Can you work these out from the drawing? Everything is in mm from the part's minimum corner. Round coordinates to 2 decimals unless told otherwise and drop trailing zeros. Loops run counter-clockwise (first coordinate to the right, second up) from the corner with the lowest first, then second, coordinate; pieces in that order, holes last. Notation, with made-up numbers: M 55.5,-9 L 86.5,-9 A15 cw 86.5,9 Z; hole C 22,48 d7. An arc over 180 degrees is marked long. Use a Markdown table: item, result.
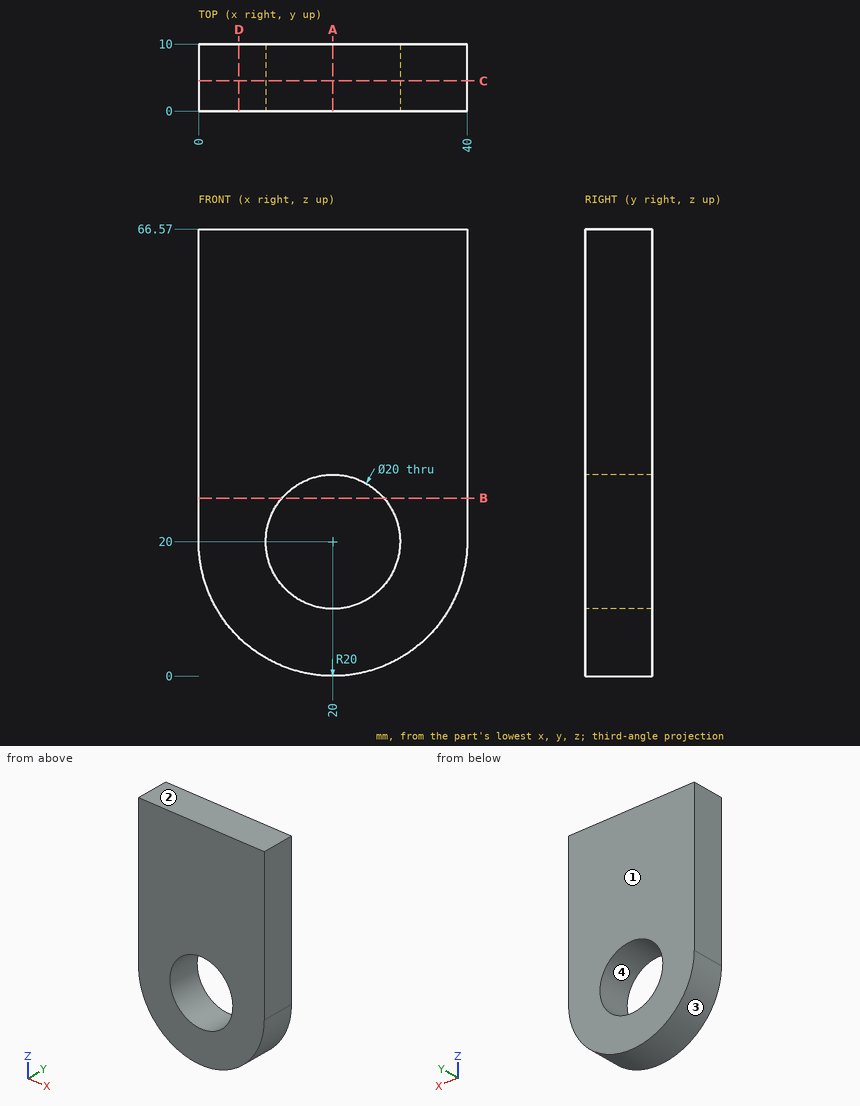
1. For pin 1 Ø1.5 at (y, z) = (2, 18.5) entering from -X; pin 2 Ø4 at (x, y) = (12.5, 6) entering from -Z, each with a flat end and sliding along its axis, tell me the tip position at first contact or that it passes through.
Answer sheet:
| item | result |
|---|---|
| pin 1 | x = 0.01 |
| pin 2 | z = 0.77 |
2. Imagine slicing it at D-D, the plane x = 6. Write out the boundary of the cut face in (y, z).
Answer sheet:
| item | result |
|---|---|
| outline | M 0,5.72 L 10,5.72 L 10,66.57 L 0,66.57 Z |
3. Imagine slicing it at B-B, the plane z = 26.5. Write out the boundary of the cut face in (x, y), then the cut area to 3 significant figures.
Answer sheet:
| item | result |
|---|---|
| outline | M 0,0 L 12.4,0 L 12.4,10 L 0,10 Z; M 27.6,0 L 40,0 L 40,10 L 27.6,10 Z |
| area | 248 mm2 |
4. Imagine slicing it at A-A, the plane x = 20. Write out the boundary of the cut face in (y, z).
Answer sheet:
| item | result |
|---|---|
| outline | M 0,0 L 10,0 L 10,10 L 0,10 Z; M 0,30 L 10,30 L 10,66.57 L 0,66.57 Z |
5. We'd pull the mould along Z, two halves only. Please class the marked faces 1, 2, 3 and 4: +Z half, -Z half, draft (parallel to the pull), parting line (faces both ways), or undercut.
Answer sheet:
| item | result |
|---|---|
| face 1 | draft |
| face 2 | +Z half |
| face 3 | -Z half |
| face 4 | undercut |
6. I need wall thicknesses on probe 1 along X at (y, z) = (6.25, 20); probe 2 along X at (y, z) = (5, 19); probe 3 along Z at (x, y) = (12, 2.5). Which ranges of each line are inside material? Lowest first, please. Write a range as from..to.
Answer sheet:
| item | result |
|---|---|
| probe 1 | 0..10, 30..40 |
| probe 2 | 0.03..10.05, 29.95..39.97 |
| probe 3 | 1.67..14, 26..66.57 |
7. Imagine slicing it at C-C, the plane y = 4.5. Write out the boundary of the cut face in (x, z).
Answer sheet:
| item | result |
|---|---|
| outline | M 0,20 A20 ccw 40,20 L 40,66.57 L 0,66.57 Z; hole C 20,20 d20 |
